The model under review builds one solid part; all positions refer to its coordinate system, in mm. Face numbers are marked on the shaded views. A direction names the side the tool comes from. Coordinates: 2 decimals unless noted, no trailing zeros. Write each loop counter-clockwise with the first axis right and the second up, starting at its lowest first coordinate (ties: lowest second). Pieces come first, ordered by that corner, then holes. Notation, with made-up numbers: (-21.75, 10.5) - (24.25, 10.5) arc R32 cw to (24.25, 49.5) - close; hole circle Ø8 at (87, 72). An arc over 180 degrees is marked (long way). Put each result on its own line as item: value. Start each with the question number.
Item 1: Consider section D-D on x = 39.5. Give the boundary of the cut face in (y, z), then the cut area to 3 significant figures.
Item 2: To check wall thickness, follow L1, parallel to Y at x = 0, z = -1.75; L2, parallel to X at y = 12.5, z = 4.75; L3, parallel to Y at x = -10.5, z = 8.75. State the ranges of each line that lie inside material, in increasing order. Write a range as [from, to].
Item 3: Consider section C-C on z = 1.25. State how many separate pieces and enclosed holes the cut face has, then the cut area to 3 significant figures.
Item 4: For pin 1 (8 mm diameter, centred on x = -46, y = -54, fed in from -Z); pin 2 (12 mm diameter, centred on x = 38, y = 8.5, fed in from +Z); pin 3 (8 mm diameter, centred on y = -28, z = -4, fed in from -X); pin 4 (6 mm diameter, centred on x = 3.5, z = 2.5, fed in from -Y), all flat-tipped, find the tip position at first contact; note any pin that passes through.
Item 5: Consider section A-A on x = 0. Give the boundary of the cut face in (y, z).
Item 6: Machinability: for the marked faces 4, 5 and 6, which of the approach directions +Z, -Z, +X, -X, +Y, -Y give a long, thin tool a straight path to every point of the face, cutting with its end or side? Answer none if there is none.
Item 7: Consider section B-B on y = -34. Give the boundary of the cut face in (x, z).
Item 8: Mouldability with a two-part tool opening along X and no side actions: class the marked faces 1, 2 and 3 as pulls with the +X half, pulls with the -X half, needs draft (parallel to the pull), parting line crosses it, or undercut.
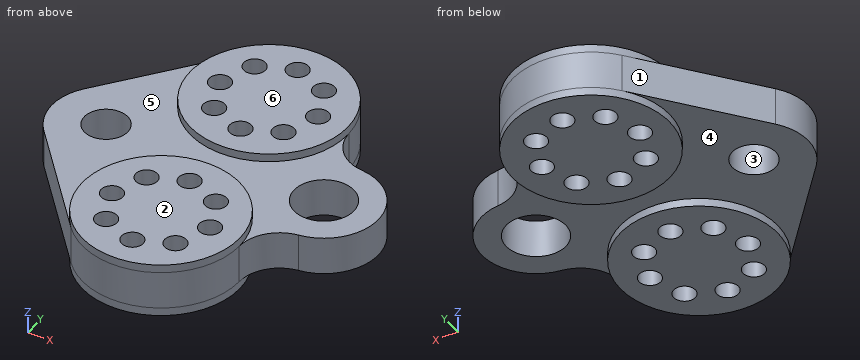
```python
from build123d import *

# Parameters (mm, degrees)
PLATE_PROFILE_SKETCH_R      = 8
PLATE_PROFILE_SKETCH_R_2    = 11
CONNECTING_PLATE_14MM_DEPTH = 7
HUB_BOSSES_SKETCH_R         = 29
HUB_BOSSES_20MM_DEPTH       = 10
BOLT_CIRCLE_HOLES_SKETCH_R  = 4
BOLT_HOLES_2X8X_8_DEPTH     = 116.797237


with BuildPart() as part:
    # Plate Profile Sketch → Connecting Plate 14mm (new, symmetric)
    with BuildSketch(Plane.XY):
        with BuildLine():
            Line((-55.373684, -21.20743), (-22.291842, 18.549226))
            ThreePointArc((-22.291842, 18.549226), (9.623005, 27.35686), (28.995542, 0.508459))
            ThreePointArc((28.995542, 0.508459), (32.885859, -9.309525), (42.281849, -14.130597))
            ThreePointArc((42.281849, -14.130597), (60, -34), (42.281849, -53.869403))
            ThreePointArc((42.281849, -53.869403), (32.885859, -58.690475), (28.995542, -68.508459))
            ThreePointArc((28.995542, -68.508459), (9.623005, -95.35686), (-22.291842, -86.549226))
            Line((-22.291842, -86.549226), (-55.373684, -46.79257))
            ThreePointArc((-55.373684, -46.79257), (-60, -34), (-55.373684, -21.20743))
        make_face()
        with Locations((-40, -34)):
            Circle(PLATE_PROFILE_SKETCH_R, mode=Mode.SUBTRACT)
        with Locations((40, -34)):
            Circle(PLATE_PROFILE_SKETCH_R_2, mode=Mode.SUBTRACT)
    extrude(amount=CONNECTING_PLATE_14MM_DEPTH, both=True)

    # Hub Bosses Sketch → Hub Bosses 20mm (add, symmetric)
    with BuildSketch(Plane.XY):
        Circle(HUB_BOSSES_SKETCH_R)
        with Locations((0, -68)):
            Circle(HUB_BOSSES_SKETCH_R)
    extrude(amount=HUB_BOSSES_20MM_DEPTH, both=True)

    # Bolt Circle Holes Sketch → Bolt Holes 2x8xØ8 (cut, through all)
    with BuildSketch(Plane.XY.offset(10)):
        with Locations((0, 18)):
            Circle(BOLT_CIRCLE_HOLES_SKETCH_R)
        with Locations((12.727922, 12.727922)):
            Circle(BOLT_CIRCLE_HOLES_SKETCH_R)
        with Locations((18, 0)):
            Circle(BOLT_CIRCLE_HOLES_SKETCH_R)
        with Locations((12.727922, -12.727922)):
            Circle(BOLT_CIRCLE_HOLES_SKETCH_R)
        with Locations((0, -18)):
            Circle(BOLT_CIRCLE_HOLES_SKETCH_R)
        with Locations((-12.727922, -12.727922)):
            Circle(BOLT_CIRCLE_HOLES_SKETCH_R)
        with Locations((-18, 0)):
            Circle(BOLT_CIRCLE_HOLES_SKETCH_R)
        with Locations((-12.727922, 12.727922)):
            Circle(BOLT_CIRCLE_HOLES_SKETCH_R)
        with Locations((0, -50)):
            Circle(BOLT_CIRCLE_HOLES_SKETCH_R)
        with Locations((12.727922, -55.272078)):
            Circle(BOLT_CIRCLE_HOLES_SKETCH_R)
        with Locations((18, -68)):
            Circle(BOLT_CIRCLE_HOLES_SKETCH_R)
        with Locations((12.727922, -80.727922)):
            Circle(BOLT_CIRCLE_HOLES_SKETCH_R)
        with Locations((0, -86)):
            Circle(BOLT_CIRCLE_HOLES_SKETCH_R)
        with Locations((-12.727922, -80.727922)):
            Circle(BOLT_CIRCLE_HOLES_SKETCH_R)
        with Locations((-18, -68)):
            Circle(BOLT_CIRCLE_HOLES_SKETCH_R)
        with Locations((-12.727922, -55.272078)):
            Circle(BOLT_CIRCLE_HOLES_SKETCH_R)
    extrude(amount=-BOLT_HOLES_2X8X_8_DEPTH, mode=Mode.SUBTRACT)


solid = part.part
```
Report:
1. outline: (-54.46, -7) - (-44.99, -7) - (-44.99, 7) - (-54.46, 7) - close; (-23.01, -7) - (-13.54, -7) - (-13.54, 7) - (-23.01, 7) - close
1. area: 265 mm²
2. L1: [-97, -90], [-82, -54], [-46, -22], [-14, 14], [22, 29]
2. L2: [-27.33, -16.72], [-8.73, 8.73], [16.72, 26.17]
2. L3: [-95.03, -84.05], [-77.41, -58.59], [-51.95, -40.97], [-27.03, -16.05], [-9.41, 9.41], [16.05, 27.03]
3. separate pieces: 1
3. enclosed holes: 18
3. area: 7,980 mm²
4. pin 1: z = -7
4. pin 2: through
4. pin 3: x = -59.9
4. pin 4: y = -97
5. outline: (-97, -10) - (-90, -10) - (-90, 10) - (-97, 10) - close; (-82, -10) - (-54, -10) - (-54, 10) - (-82, 10) - close; (-46, -10) - (-39, -10) - (-39, -7) - (-29, -7) - (-29, -10) - (-22, -10) - (-22, 10) - (-29, 10) - (-29, 7) - (-39, 7) - (-39, 10) - (-46, 10) - close; (-14, -10) - (14, -10) - (14, 10) - (-14, 10) - close; (22, -10) - (29, -10) - (29, 10) - (22, 10) - close
6. face 4: -Z
6. face 5: +Z
6. face 6: +Z, +X, -X, +Y, -Y
7. outline: (-60, -7) - (-48, -7) - (-48, 7) - (-60, 7) - close; (-32, -7) - (29, -7) - (29, 7) - (-32, 7) - close; (51, -7) - (60, -7) - (60, 7) - (51, 7) - close
8. face 1: pulls with the -X half
8. face 2: needs draft
8. face 3: undercut
